For this review, take the finished solid that the model builds, in its own axes (mm). A direction names the side the tool comes from. Round coordinates to 2 decimals unless told otherwise and drop trailing zeros. Write each loop counter-clockwise with the first axis right and the second up, starting at its lowest first coordinate (ties: lowest second). Pieces come first, ordered by that corner, then holes. Notation, with made-up numbers: (62, 84) - (73, 84) arc R15 cw to (73, 101) - close; hole circle Ø9 at (42, 18.25). An arc over 180 degrees is marked (long way). Answer in a Markdown table with one row per item. Add a question column.
from build123d import *

# Parameters (mm, degrees)
SKETCH1_W                                           = 142
SKETCH1_H                                           = 100
EXTRUDE1_DEPTH                                      = 12
CBORE_FOR_M5_HEX_SOCKET_HEAD_CAP_SCREW1_D           = 5.5
CBORE_FOR_M5_HEX_SOCKET_HEAD_CAP_SCREW1_CBORE_D     = 10
CBORE_FOR_M5_HEX_SOCKET_HEAD_CAP_SCREW1_CBORE_DEPTH = 5.4
CBORE_FOR_M5_HEX_SOCKET_HEAD_CAP_SCREW2_D           = 5.5
CBORE_FOR_M5_HEX_SOCKET_HEAD_CAP_SCREW2_CBORE_D     = 10
CBORE_FOR_M5_HEX_SOCKET_HEAD_CAP_SCREW2_CBORE_DEPTH = 5.4
MM_0_D                                              = 4
CHAMFER1_SIZE                                       = 12
F_4_0_MM_DOWEL_HOLES1_D                             = 4
F_8_0_MM_DOWEL_HOLES1_D                             = 8
SKETCH13_R                                          = 7
EXTRUDE2_DEPTH                                      = 7
F_4_0_MM_DOWEL_HOLES2_D                             = 4


with BuildPart() as part:
    # Sketch1 → Extrude1 (new body)
    with BuildSketch(Plane(origin=(0, 0, 0), x_dir=(1, 0, 0), z_dir=(0, 1, 0))):
        Rectangle(SKETCH1_W, SKETCH1_H)
    extrude(amount=EXTRUDE1_DEPTH)

    # CBORE for M5 Hex Socket Head Cap Screw1 (through all)
    with Locations(Plane(origin=(0, 0, 0), x_dir=(-1, 0, 0), z_dir=(0, -1, 0))):
        with Locations((-13, -39), (13, 39), (-13, 39), (13, -39)):
            CounterBoreHole(CBORE_FOR_M5_HEX_SOCKET_HEAD_CAP_SCREW1_D / 2, CBORE_FOR_M5_HEX_SOCKET_HEAD_CAP_SCREW1_CBORE_D / 2, CBORE_FOR_M5_HEX_SOCKET_HEAD_CAP_SCREW1_CBORE_DEPTH)

    # CBORE for M5 Hex Socket Head Cap Screw2 (through all)
    with Locations(Plane(origin=(0, 12, 0), x_dir=(1, 0, 0), z_dir=(0, 1, 0))):
        with Locations((-54, 0), (54, 0), (-18, 0), (18, 0)):
            CounterBoreHole(CBORE_FOR_M5_HEX_SOCKET_HEAD_CAP_SCREW2_D / 2, CBORE_FOR_M5_HEX_SOCKET_HEAD_CAP_SCREW2_CBORE_D / 2, CBORE_FOR_M5_HEX_SOCKET_HEAD_CAP_SCREW2_CBORE_DEPTH)

    # 大小mm 暗销孔0 (through all)
    with Locations(Plane(origin=(0, 12, 0), x_dir=(1, 0, 0), z_dir=(0, 1, 0))):
        with Locations((-40, 27), (40, 27), (40, -27), (-40, -27)):
            Hole(MM_0_D / 2)

    # Chamfer1
    chamfer1_edges = [part.edges().sort_by_distance(p)[0] for p in [
        (-71, 6, -50),
        (71, 6, -50),
        (71, 6, 50),
        (-71, 6, 50),
    ]]
    chamfer(chamfer1_edges, length=CHAMFER1_SIZE)

    # Ø4.0 mm Dowel Holes1 (through all)
    with Locations(Plane(origin=(0, 12, 0), x_dir=(1, 0, 0), z_dir=(0, 1, 0))):
        with Locations((-65, 0), (65, 0)):
            Hole(F_4_0_MM_DOWEL_HOLES1_D / 2)

    # Ø8.0 mm Dowel Holes1 (through all)
    with Locations(Plane(origin=(0, 12, 0), x_dir=(1, 0, 0), z_dir=(0, 1, 0))):
        with Locations((-42, 42.5), (42, 42.5), (42, -42.5), (-42, -42.5)):
            Hole(F_8_0_MM_DOWEL_HOLES1_D / 2)

    # Sketch13 → Extrude2 (cut)
    with BuildSketch(Plane(origin=(0, 12, 0), x_dir=(1, 0, 0), z_dir=(0, 1, 0))):
        with Locations(Location((-42, -42.5, 0), (0, 0, 270))):
            Circle(SKETCH13_R)
        with Locations(Location((42, -42.5, 0), (0, 0, 270))):
            Circle(SKETCH13_R)
        with Locations(Location((-42, 42.5, 0), (0, 0, 270))):
            Circle(SKETCH13_R)
        with Locations(Location((42, 42.5, 0), (0, 0, 270))):
            Circle(SKETCH13_R)
    extrude(amount=-EXTRUDE2_DEPTH, mode=Mode.SUBTRACT)

    # Ø4.0 mm Dowel Holes2 (through all)
    with Locations(Plane(origin=(0, 0, 0), x_dir=(-1, 0, 0), z_dir=(0, -1, 0))):
        with Locations((0, 17), (0, -17)):
            Hole(F_4_0_MM_DOWEL_HOLES2_D / 2)


solid = part.part
Q1. To check wall thickness, follow probe 1 along Z at (x, y) = (0, 7.25); probe 2 along Z at (x, y) = (17.5, 10); probe 3 along Z at (x, y) = (54, 3.75). State the ranges of each line that lie inside material, in increasing order.
Q2. Add section D-D on y = 8. Count the separate pieces of the cut face and the enclosed holes in it, then the cut area to 3 significant figures.
Q3. Add section B-B on z = -17. State the section outline as (x, y) points, then the cut area to 3 significant figures.
Q4. Add section A-A on x = 0. State the section outline as (y, z) points.
Q5. Add section C-C on x = -54. State the section outline as (y, z) points.
Q6. Insertion check: pin 1 Ø3.5 at (x, z) = (65, 0) entering from -Y; pin 2 Ø7 at (x, z) = (-13, -39) entering from -Y; pin 3 Ø8 at (x, z) = (-19, 0.5) entering from +Y; pin 4 Ø3 at (x, z) = (52, 0.5) entering from +Y. Each pin has a flat end and moves straight along its axis. Give the tip position at first contact, or say it passes through.
Q7. Tool access review of faces 1 (the face through (-16, 3, 35)), 2 (the face through (-13.358, 8.746, -41.727)), 3 (the face through (47.902, 8.549, 46.263)): name each direction out of +Z, -Z, +X, -X, +Y, -Y from which nothing blocks a thin tool from reaching the whole face with its end or side.
Answer sheet:
| question | item | result |
|---|---|---|
| 1 | probe 1 | z = -50 to -19, -15 to 15, 19 to 50 |
| 1 | probe 2 | z = -50 to -4.97, 4.97 to 50 |
| 1 | probe 3 | z = -50 to -2.75, 2.75 to 50 |
| 2 | separate pieces | 1 |
| 2 | enclosed holes | 20 |
| 2 | area | 12,800 mm² |
| 3 | outline | (-71, 0) - (-2, 0) - (-2, 12) - (-71, 12) - close; (2, 0) - (71, 0) - (71, 12) - (2, 12) - close |
| 3 | area | 1,660 mm² |
| 4 | outline | (0, -50) - (12, -50) - (12, -19) - (0, -19) - close; (0, -15) - (12, -15) - (12, 15) - (0, 15) - close; (0, 19) - (12, 19) - (12, 50) - (0, 50) - close |
| 5 | outline | (0, -50) - (12, -50) - (12, -5) - (6.6, -5) - (6.6, -2.75) - (0, -2.75) - close; (0, 2.75) - (6.6, 2.75) - (6.6, 5) - (12, 5) - (12, 50) - (0, 50) - close |
| 6 | pin 1 | passes through |
| 6 | pin 2 | stops at y = 5.4 |
| 6 | pin 3 | stops at y = 12 |
| 6 | pin 4 | stops at y = 6.6 |
| 7 | face 1 | -Y |
| 7 | face 2 | +Y, -Y |
| 7 | face 3 | +Y |
